from build123d import *


with BuildPart() as part:
    # Bush Half-Section Profile → Flanged Bush Body (revolve)
    with BuildSketch(Plane.XY, mode=Mode.PRIVATE) as flanged_bush_body_sk:
        Polygon((12, 0), (12, 16.5), (16.5, 21), (21, 21), (21, 15), (16.5, 15), (16.5, 0), align=None)
    revolve(flanged_bush_body_sk.sketch.rotate(Axis((0, 0, 0), (0, 1, 0)), 90), axis=Axis((0, 0, 0), (0, 1, 0)))


solid = part.part
CAD build for the part. Positions are in the model's coordinates, mm. Coordinates: 2 decimals unless noted, no trailing zeros. Write each loop counter-clockwise with the first axis right and the second up, starting at its lowest first coordinate (ties: lowest second). Pieces come first, ordered by that corner, then holes. Notation, with made-up numbers: M -5.5,-5.5 L 53.5,-5.5 A25 cw 53.5,10.5 Z; hole C 75.5,-28 d8. An arc over 180 degrees is marked long. Answer as a JSON object with one key per item and string values. Group by question number.
1) Pin check, flat tips, straight feed: pin 1 Ø6 at (y, z) = (10, -1.5) entering from -X; pin 2 Ø1 at (y, z) = (15, -14.5) entering from +X; pin 3 Ø10 at (x, y) = (-5.5, 4.5) entering from +Z. Stop position of each tip, or through.
2) Saw through at A-A (x = 0). Write the cut outline in (y, z), plus the area to 3 significant figures.
3) Wall check: line 1 (X direction, y = 10, z = 0); line 2 (Y direction, x = 15.5, z = 10.5); line 3 (X direction, y = 5.75, z = -4.5). Give the ranges that are in metal, low to high. Write a range as from..to.
4) Saw through at C-C (y = 9.75). Write the cut outline in (x, z), plus the area to 3 significant figures.
5) Mould opens along X. For faces 1 (the face through (11, 15, 13)), 2 (the face through (7.47, 16.78, 9.75)), 3 (the face through (-4.956, 7.395, -15.738)), 4 (the face through (-3.604, 8.366, -11.446)) say: +X half, -X half, draft (parallel to the pull), parting line (faces both ways), or undercut.
6) Saw through at B-B (z = 0). Write the cut outline in (x, y).
7) Saw through at D-D (z = 18.5). Write the cut outline in (x, y), plus the area to 3 significant figures.
Values follow:
{
 "1": {"pin 1": "stops at x = -16.5", "pin 2": "stops at x = 15.65", "pin 3": "stops at z = 16.49"},
 "2": {"outline": "M 0,-16.5 L 15,-16.5 L 15,-21 L 21,-21 L 21,-16.5 L 16.5,-12 L 0,-12 Z; M 0,12 L 16.5,12 L 21,16.5 L 21,21 L 15,21 L 15,16.5 L 0,16.5 Z", "area": "223 mm2"},
 "3": {"line 1": "x = -16.5..-12, 12..16.5", "line 2": "y = 15..21", "line 3": "x = -15.87..-11.12, 11.12..15.87"},
 "4": {"outline": "C 0,0 d33; hole C 0,0 d24", "area": "403 mm2"},
 "5": {"face 1": "draft", "face 2": "undercut", "face 3": "parting line", "face 4": "undercut"},
 "6": {"outline": "M -21,15 L -16.5,15 L -16.5,0 L -12,0 L -12,16.5 L -16.5,21 L -21,21 Z; M 12,0 L 16.5,0 L 16.5,15 L 21,15 L 21,21 L 16.5,21 L 12,16.5 Z"},
 "7": {"outline": "M -9.94,15 L 9.94,15 L 9.94,21 L -9.94,21 Z", "area": "119 mm2"}
}
